from build123d import *

# Parameters (mm, degrees)
SKETCH1_W                  = 20
SKETCH1_H                  = 43
BOSS_EXTRUDE1_DEPTH        = 50
SKETCH2_R                  = 15
CUT_EXTRUDE1_DEPTH         = 50
CUT_EXTRUDE2_DEPTH         = 5
SKETCH4_W                  = 6
SKETCH4_H                  = 5
CUT_EXTRUDE3_DEPTH         = 3
SIZE_MM_DOWEL_HOLE_1_D     = 4.2
SIZE_MM_DOWEL_HOLE_1_DEPTH = 14.2
SIZE_MM_DOWEL_HOLE_1_TIP   = 1.2618073
SKETCH8_W                  = 10
SKETCH8_H                  = 40
CUT_EXTRUDE4_DEPTH         = 3
SIZE_MM_DOWEL_HOLE_2_D     = 5
SIZE_MM_DOWEL_HOLE_2_DEPTH = 17.1
SIZE_MM_DOWEL_HOLE_2_TIP   = 1.502151548


with BuildPart() as part:
    # Sketch1 → Boss-Extrude1 (new body)
    with BuildSketch(Plane.XY):
        Rectangle(SKETCH1_W, SKETCH1_H)
    extrude(amount=BOSS_EXTRUDE1_DEPTH)

    # Sketch2 → Cut-Extrude1 (cut)
    with BuildSketch(Plane(origin=(10, 0, 0), x_dir=(0, 0, -1), z_dir=(1, 0, 0))):
        with Locations((-25, -21.5)):
            Circle(SKETCH2_R)
    extrude(amount=-CUT_EXTRUDE1_DEPTH, mode=Mode.SUBTRACT)

    # Sketch3 → Cut-Extrude2 (cut)
    with BuildSketch(Plane.ZY.offset(10)):
        with BuildLine():
            Line((19.083920217, -4.5), (30.916079783, -4.5))
            ThreePointArc((30.916079783, -4.5), (25, -39.5), (19.083920217, -4.5))
        make_face()
    extrude(amount=-CUT_EXTRUDE2_DEPTH, mode=Mode.SUBTRACT)

    # Sketch4 → Cut-Extrude3 (cut)
    with BuildSketch(Plane.XZ.offset(21.5)):
        with Locations((0, 2.5)):
            Rectangle(SKETCH4_W, SKETCH4_H)
        with Locations((0, 47.5)):
            Rectangle(SKETCH4_W, SKETCH4_H)
    extrude(amount=-CUT_EXTRUDE3_DEPTH, mode=Mode.SUBTRACT)

    # Size mm Dowel hole 1
    with Locations(Plane(origin=(0, -21.5, 0), x_dir=(-1, 0, 0), z_dir=(0, -1, 0))):
        with Locations((6, -4), (-6, -4), (6, -46), (-6, -46)):
            Hole(SIZE_MM_DOWEL_HOLE_1_D / 2, depth=SIZE_MM_DOWEL_HOLE_1_DEPTH)
            with Locations((0, 0, -(SIZE_MM_DOWEL_HOLE_1_DEPTH + SIZE_MM_DOWEL_HOLE_1_TIP / 2))):  # 118° drill point
                Cone(0, SIZE_MM_DOWEL_HOLE_1_D / 2, SIZE_MM_DOWEL_HOLE_1_TIP, mode=Mode.SUBTRACT)

    # Sketch8 → Cut-Extrude4 (cut)
    with BuildSketch(Plane(origin=(0, 21.5, 0), x_dir=(1, 0, 0), z_dir=(0, 1, 0))):
        with Locations((0, -25)):
            Rectangle(SKETCH8_W, SKETCH8_H)
    extrude(amount=-CUT_EXTRUDE4_DEPTH, mode=Mode.SUBTRACT)

    # Size mm Dowel hole 2
    with Locations(Plane(origin=(0, 18.5, 0), x_dir=(1, 0, 0), z_dir=(0, 1, 0))):
        with Locations((0, -13), (0, -37)):
            Hole(SIZE_MM_DOWEL_HOLE_2_D / 2, depth=SIZE_MM_DOWEL_HOLE_2_DEPTH)
            with Locations((0, 0, -(SIZE_MM_DOWEL_HOLE_2_DEPTH + SIZE_MM_DOWEL_HOLE_2_TIP / 2))):  # 118° drill point
                Cone(0, SIZE_MM_DOWEL_HOLE_2_D / 2, SIZE_MM_DOWEL_HOLE_2_TIP, mode=Mode.SUBTRACT)


solid = part.part
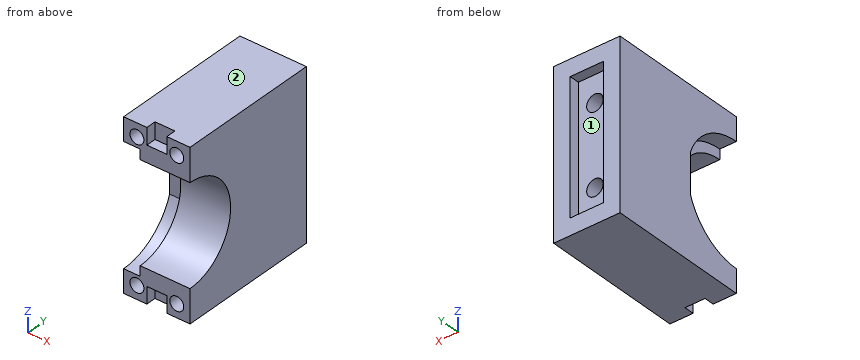
Geometry check sheet. Reference: the model listing, model coordinates, mm. Face numbers are marked on the shaded views. A direction names the side the tool comes from. Round coordinates to 2 decimals unless told otherwise and drop trailing zeros. Loops run counter-clockwise (first coordinate to the right, second up) from the corner with the lowest first, then second, coordinate; pieces in that order, holes last. Notation, with made-up numbers: (83, 50.5) - (91, 50.5) arc R13 ccw to (91, 66.5) - close; hole circle Ø3 at (73, 69.25). An arc over 180 degrees is marked (long way). One line per question, with ' | ' between items. Start each with the question number.
1. Tool access check on the marked faces 1 and 2. Record the directions out of +Z, -Z, +X, -X, +Y, -Y that give a thin tool (end or side, any length) a straight path to the whole face; none if there is none.
2. Cross-section at A-A on y = -13. Record the cut outline in (x, z).
3. Cross-section at B-B on z = 25. Record the cut outline in (x, y).
4. Scan lines: line 1 (X direction, y = -12, z = 46); line 2 (Z direction, x = 0, y = 8); line 3 (Z direction, x = 6, y = -14.25). Record each from-to range of solid material in increasing order. Write a range as [from, to].
5. Depth check by flat-ended pin: pin 1 (2.5 mm diameter, centred on x = -1.5, z = 48.5, fed in from -Y); pin 2 (2.5 mm diameter, centred on x = -6.5, z = 27, fed in from -Y); pin 3 (6 mm diameter, centred on x = -1, z = 30, fed in from +Y). Enter the tip coordinate at first touch or a pass-through.
Taken from the geometry:
1) face 1: +Y | face 2: +Z, +X, -X, +Y, -Y
2) outline: (-10, 0) - (10, 0) - (10, 12.64) - (-5, 12.64) - (-5, 9.13) - (-10, 9.13) - close; (-10, 40.87) - (-5, 40.87) - (-5, 37.36) - (10, 37.36) - (10, 50) - (-10, 50) - close; hole circle Ø4.2 at (-6, 4); hole circle Ø4.2 at (-6, 46); hole circle Ø4.2 at (6, 4); hole circle Ø4.2 at (6, 46)
3) outline: (-10, -4.5) - (-5, -4.5) - (-5, -6.5) - (10, -6.5) - (10, 21.5) - (5, 21.5) - (5, 18.5) - (-5, 18.5) - (-5, 21.5) - (-10, 21.5) - close
4) line 1: [-10, -8.1], [-3.9, 3.9], [8.1, 10] | line 2: [0, 10.5], [15.5, 34.5], [39.5, 50] | line 3: [0, 1.9], [6.1, 11.87], [38.13, 43.9], [48.1, 50]
5) pin 1: y = -18.5 | pin 2: y = -4.5 | pin 3: y = 18.5
